Verification items for this drawing (mm, ordinates from the low corner). A direction names the side the tool comes from. Coordinates: 2 decimals unless noted, no trailing zeros. Order: outer loops, then holes, each group sorted by start corner. A loop starts at its lowest first (then second) coordinate and runs counter-clockwise, first axis right, second up. Notation, with made-up numbers: M 10,-16 L 32,-16 A8 ccw 32,-12 Z; hole C -38.5,-5.75 d8. An arc over 180 degrees is marked long. Use CSV: the item, a comma, the result in double quotes. Start each with the question number.
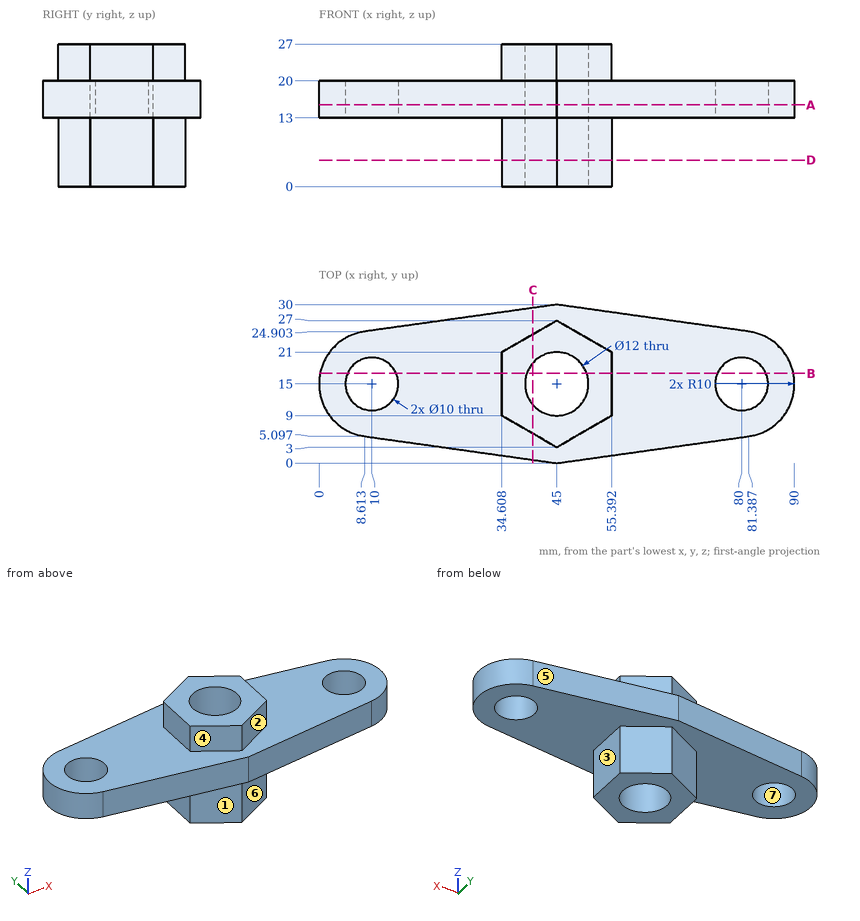
1) Section check A-A on z = 15.5. Record the boundary of the cut face in (x, y).
2) Gauge pin test, flat ends, axial feed: P1, Ø1, axis at x = 30, y = 23, coming from the +Z side; P2, Ø9, axis at x = 27.5, y = 17, coming from the -Z side; P3, Ø15.5, axis at x = 45, y = 15, coming from the +Z side; P4, Ø10, axis at y = 20.5, z = 19.5, coming from the -X side. Record the tip position at first contact, or that the pin passes through.
3) Set-up check for the marked faces 1, 2, 3 and 4: record each of +Z, -Z, +X, -X, +Y, -Y from which the full face is reachable in a straight line by a thin tool's end or side.
4) Section check C-C on x = 40.5. Record the boundary of the cut face in (y, z).
5) Draft check along Y on the marked faces 5, 6 and 7. Enter one of: +Y half, -Y half, draft (parallel to the pull), parting line (faces both ways), or undercut.
6) Material ranges on line 1 along Y through (x, z) = (45, 12); line 2 along Z through (x, y) = (56, 20.75); line 3 along Y through (x, z) = (10, 16), recorded low to high.
7) Section check B-B on y = 17. Record the boundary of the cut face in (x, z), then the cut area to 3 significant figures.
8) Section check D-D on z = 5. Record the boundary of the cut face in (x, y), then the cut area to 3 significant figures.
Results are:
1,outline,"M 8.61,5.1 L 45,0 L 81.39,5.1 A10 ccw 81.39,24.9 L 45,30 L 8.61,24.9 A10 ccw Z; hole C 10,15 d10; hole C 45,15 d12; hole C 80,15 d10"
2,P1,"stops at z = 20"
2,P2,"stops at z = 13"
2,P3,"stops at z = 27"
2,P4,"stops at x = 0.01"
3,face 1,"-Z, -X, -Y"
3,face 2,"+Z, +X, -Y"
3,face 3,"-Z, +X, +Y, -Y"
3,face 4,"+Z, -X, -Y"
4,outline,"M 0.63,13 L 5.6,13 L 5.6,0 L 11.03,0 L 11.03,27 L 5.6,27 L 5.6,20 L 0.63,20 Z; M 18.97,0 L 24.4,0 L 24.4,13 L 29.37,13 L 29.37,20 L 24.4,20 L 24.4,27 L 18.97,27 Z"
5,face 5,"+Y half"
5,face 6,"-Y half"
5,face 7,"undercut"
6,line 1,"y = 3 to 9, 21 to 27"
6,line 2,"z = 13 to 20"
6,line 3,"y = 4.9 to 10, 20 to 25.1"
7,outline,"M 0.2,13 L 5.42,13 L 5.42,20 L 0.2,20 Z; M 14.58,13 L 34.61,13 L 34.61,0 L 39.34,0 L 39.34,27 L 34.61,27 L 34.61,20 L 14.58,20 Z; M 50.66,0 L 55.39,0 L 55.39,13 L 75.42,13 L 75.42,20 L 55.39,20 L 55.39,27 L 50.66,27 Z; M 84.58,13 L 89.8,13 L 89.8,20 L 84.58,20 Z"
7,area,"609 mm²"
8,outline,"M 34.61,9 L 45,3 L 55.39,9 L 55.39,21 L 45,27 L 34.61,21 Z; hole C 45,15 d12"
8,area,"261 mm²"
